```python
from build123d import *

# Parameters (mm, degrees)
SKETCH_1_W          = 46.4
SKETCH_1_H          = 15.6
SKETCH_1_R          = 1.6
EXTRUDE_1_DEPTH     = 1.5
SKETCH_2_R          = 23
CUT_EXTRUDE_1_DEPTH = 45.229515032
CUT_EXTRUDE_2_DEPTH = 45.229515032
FILLET_1_R          = 2


with BuildPart() as part:
    # 草图1 → 凸台-拉伸1 (new body)
    with BuildSketch(Plane(origin=(0, 0, 0), x_dir=(0, 0, -1), z_dir=(1, 0, 0))):
        with Locations((19.4, -4)):
            Rectangle(SKETCH_1_W, SKETCH_1_H)
        Circle(SKETCH_1_R, mode=Mode.SUBTRACT)
        with Locations((0, -8)):
            Circle(SKETCH_1_R, mode=Mode.SUBTRACT)
        with Locations((38.8, 0)):
            Circle(SKETCH_1_R, mode=Mode.SUBTRACT)
        with Locations((38.8, -8)):
            Circle(SKETCH_1_R, mode=Mode.SUBTRACT)
    extrude(amount=EXTRUDE_1_DEPTH)

    # 草图2 → 切除-拉伸1 (cut, through all)
    with BuildSketch(Plane(origin=(1.5, 0, 0), x_dir=(0, 0, -1), z_dir=(1, 0, 0))):
        with Locations((19.4, -34)):
            Circle(SKETCH_2_R)
    extrude(amount=-CUT_EXTRUDE_1_DEPTH, mode=Mode.SUBTRACT)

    # 草图3 → 切除-拉伸2 (cut, through all)
    with BuildSketch(Plane(origin=(1.5, 0, 0), x_dir=(0, 0, -1), z_dir=(1, 0, 0))):
        with BuildLine():
            Line((6, -0.2), (32.8, -0.2))
            Line((32.8, -0.2), (32.8, -7.8))
            Line((32.8, -7.8), (25.413318551, -7.8))
            ThreePointArc((25.413318551, -7.8), (19.4, -7), (13.386681449, -7.8))
            Line((13.386681449, -7.8), (6, -7.8))
            Line((6, -7.8), (6, -0.2))
        make_face()
    extrude(amount=-CUT_EXTRUDE_2_DEPTH, mode=Mode.SUBTRACT)

    # 圆角1
    fillet_1_edges = [part.edges().sort_by_distance(p)[0] for p in [
        (0.75, -11.8, -25.413318551),
        (0.75, -11.8, -13.386681449),
        (0.75, -7.8, -6),
        (0.75, -0.2, -6),
        (0.75, -0.2, -32.8),
        (0.75, -7.8, -32.8),
        (0.75, -7.8, -25.413318551),
        (0.75, -7.8, -13.386681449),
        (0.75, 3.8, 3.8),
        (0.75, 3.8, -42.6),
        (0.75, -11.8, -42.6),
        (0.75, -11.8, 3.8),
    ]]
    fillet(fillet_1_edges, radius=FILLET_1_R)


solid = part.part
```
CAD build for the part. Positions are in the model's coordinates, mm. A direction names the side the tool comes from. Give positions to 0.01 mm unless a question says otherwise; leave off trailing zeros. Write each loop counter-clockwise with the first axis right and the second up, starting at its lowest first coordinate (ties: lowest second). Pieces come first, ordered by that corner, then holes. Notation, with made-up numbers: M 31,89.25 L 50,89.25 A38 ccw 50,127.25 Z; hole C 73.25,27.25 d3. An arc over 180 degrees is marked long. Return JSON: item names as keys, results as strings. Group by question number.
(1) Band-saw the part on D-D (y = -9). Give the cut face in (x, z), and give its area (3 significant figures).
(2) Mould opens along Z. For faces 1 (the face through (1, 3.8, -19)), 2 (the face through (1, -7.8, -28)), 3 (the face through (1, -4, 3.8)) say: pulls with the +Z half, pulls with the -Z half, needs draft (parallel to the pull), parting line crosses it, or undercut.
(3) Drill centre lines: L1, parallel to Y at x = 1.2, z = 0; L2, parallel to Z at x = 0.3, y = -6; L3, parallel to Z at x = 0.55, y = 0.25. Where is each one in solid material? Low to high. Write a range as [from, to].
(4) Band-saw the part on C-C (z = -9.5). Give the cut face in (x, y), and give its area (3 significant figures).
(5) 3-axis set-ups, long thin cutter, end or side, ignore diameter. For faces 4 (the face through (0.76, 3.2, 3.23)), 5 (the face through (1, -7.8, -11)): which of +Z, -Z, +X, -X, +Y, -Y reach the whole face in a straight line?
(6) Band-saw the part on A-A (z = 0). Give the cut face in (x, y), and give its area (3 significant figures).
(7) Band-saw the part on B-B (x = 0.65). Give the cut face in (y, z).
Entries:
{
 "1": {"outline": "M 0,-42.6 L 1.5,-42.6 L 1.5,-40.05 L 0,-40.05 Z; M 0,-37.55 L 1.5,-37.55 L 1.5,-1.25 L 0,-1.25 Z; M 0,1.25 L 1.5,1.25 L 1.5,3.8 L 0,3.8 Z", "area": "62.1 mm^2"},
 "2": {"face 1": "needs draft", "face 2": "undercut", "face 3": "pulls with the +Z half"},
 "3": {"L1": "y = [-11.8, -9.6], [-6.4, -1.6], [1.6, 3.8]", "L2": "z = [-42.6, -32.79], [-6.01, 3.8]", "L3": "z = [-42.6, -40.38], [-37.22, -1.58], [1.58, 3.8]"},
 "4": {"outline": "M 0,-11.8 L 1.5,-11.8 L 1.5,-7.8 L 0,-7.8 Z; M 0,-0.2 L 1.5,-0.2 L 1.5,3.8 L 0,3.8 Z", "area": "12.0 mm^2"},
 "5": {"face 4": "+Z, +X, -X, +Y", "face 5": "+X, -X"},
 "6": {"outline": "M 0,-11.8 L 1.5,-11.8 L 1.5,-9.6 L 0,-9.6 Z; M 0,-6.4 L 1.5,-6.4 L 1.5,-1.6 L 0,-1.6 Z; M 0,1.6 L 1.5,1.6 L 1.5,3.8 L 0,3.8 Z", "area": "13.8 mm^2"},
 "7": {"outline": "M -11.8,-40.6 A2 ccw -9.8,-42.6 L 1.8,-42.6 A2 ccw 3.8,-40.6 L 3.8,1.8 A2 ccw 1.8,3.8 L -9.8,3.8 A2 ccw -11.8,1.8 L -11.8,-13.13 A2 ccw -11.74,-13.63 A23 cw -11.74,-25.17 A2 ccw -11.8,-25.67 Z; hole C -8,-38.8 d3.2; hole C -8,0 d3.2; hole M -7.8,-30.8 A2 ccw -5.8,-32.8 L -2.2,-32.8 A2 ccw -0.2,-30.8 L -0.2,-8 A2 ccw -2.2,-6 L -5.8,-6 A2 ccw -7.8,-8 L -7.8,-13.13 A2 ccw -7.74,-13.63 A23 cw -7.74,-25.17 A2 ccw -7.8,-25.67 Z; hole C 0,-38.8 d3.2; hole C 0,0 d3.2"}
}
